Could you check a few things on this model? Use its own coordinates, in mm. A direction names the side the tool comes from. Round coordinates to 2 decimals unless told otherwise and drop trailing zeros. Loops run counter-clockwise (first coordinate to the right, second up) from the corner with the lowest first, then second, coordinate; pieces in that order, holes last. Notation, with made-up numbers: (22.5, 35.5) -> (61.5, 35.5) arc R25 ccw to (61.5, 74.5) -> close; hole circle Ø6 at (4, 80). An arc over 180 degrees is marked (long way). Use CSV: the item, a comma, the result in double quotes. Start each with the question number.
```python
from build123d import *

# Parameters (mm, degrees)
CARRIAGE_PLATE_PROFILE_R   = 5
CARRIAGE_PLATE_PROFILE_R_2 = 3
CARRIAGE_PLATE_5MM_DEPTH   = 5


with BuildPart() as part:
    # Carriage Plate Profile → Carriage Plate 5mm (new body)
    with BuildSketch(Plane.XY):
        with BuildLine():
            Line((-10, -5), (-10, 35))
            ThreePointArc((-10, 35), (-8.535533906, 38.535533906), (-5, 40))
            Line((-5, 40), (5, 40))
            ThreePointArc((5, 40), (8.535533906, 38.535533906), (10, 35))
            Line((10, 35), (10, 30))
            Line((10, 30), (30, 30))
            ThreePointArc((30, 30), (50.922837109, 16.451383494), (75, 10))
            Line((75, 10), (80, 10))
            ThreePointArc((80, 10), (83.535533906, 8.535533906), (85, 5))
            Line((85, 5), (85, -5))
            ThreePointArc((85, -5), (83.535533906, -8.535533906), (80, -10))
            Line((80, -10), (75, -10))
            Line((75, -10), (70, -10))
            ThreePointArc((70, -10), (66.464466094, -8.535533906), (65, -5))
            Line((65, -5), (65, -4))
            ThreePointArc((65, -4), (63.828427125, -1.171572875), (61, 0))
            Line((61, 0), (14, 0))
            ThreePointArc((14, 0), (11.171572875, -1.171572875), (10, -4))
            Line((10, -4), (10, -5))
            ThreePointArc((10, -5), (8.535533906, -8.535533906), (5, -10))
            Line((5, -10), (-5, -10))
            ThreePointArc((-5, -10), (-8.535533906, -8.535533906), (-10, -5))
        make_face()
        Circle(CARRIAGE_PLATE_PROFILE_R, mode=Mode.SUBTRACT)
        with Locations((75, 0)):
            Circle(CARRIAGE_PLATE_PROFILE_R, mode=Mode.SUBTRACT)
        with Locations((0, 30)):
            Circle(CARRIAGE_PLATE_PROFILE_R_2, mode=Mode.SUBTRACT)
    extrude(amount=CARRIAGE_PLATE_5MM_DEPTH)


solid = part.part
```
1. We'd pull the mould along Y, two halves only. Please class faces 4 (the face through (-1.08, -4.88, 2.46)), 5 (the face through (20, 30, 2)), 6 (the face through (11.203, -1.141, 2.465)): pulls with the +Y half, pulls with the -Y half, needs draft (parallel to the pull), parting line crosses it, or undercut.
2. If I drill on L1, parallel to Y at x = 0, z = 1.25; L2, parallel to X at y = 3, z = 3.3; L3, parallel to X at y = 3.5, z = 0.75, over which ranges is the centre line in solid material (lowest first)?
3. Suppose I cut it at D-D (x = 33.5). List the corners of the cut face in (y, z) for me, then the cut area to 3 significant figures.
4. For faces 1 (the face through (10, 33, 2)), 2 (the face through (38, 0, 2)), 3 (the face through (-10, 15, 2)), which set-ups out of +Z, -Z, +X, -X, +Y, -Y let a thin tool reach every point of the face, with its end or its side?
5. Will these pins go through, and if not, where does the flat tip stop? pin 1 (1.5 mm diameter, centred on y = 32.5, z = 2, fed in from +X); pin 2 (3 mm diameter, centred on x = 5, y = 24.5, fed in from -Z); pin 3 (1.5 mm diameter, centred on x = 77.5, z = 3, fed in from +Y); pin 4 (2.5 mm diameter, centred on x = 25, z = 2, fed in from +Y).
6. Suppose I cut it at A-A (x = 0). List the corners of the cut face in (y, z) for me, then the cut area to 3 significant figures.
7. Suppose I cut it at B-B (z = 1.7). List the corners of the cut face in (x, y) for me, then the cut area to 3 significant figures.
8. Suppose I cut it at C-C (y = 12). List the corners of the cut face in (x, z) for me.
Geometry check:
1,face 4,"undercut"
1,face 5,"pulls with the +Y half"
1,face 6,"pulls with the -Y half"
2,L1,"y = -10 to -5, 5 to 27, 33 to 40"
2,L2,"x = -10 to -4, 4 to 71, 79 to 85"
2,L3,"x = -10 to -3.57, 3.57 to 71.43, 78.57 to 85"
3,outline,"(0, 0) -> (27.04, 0) -> (27.04, 5) -> (0, 5) -> close"
3,area,"135 mm²"
4,face 1,"+Z, -Z, +X, +Y"
4,face 2,"+Z, -Z, -Y"
4,face 3,"+Z, -Z, -X, +Y, -Y"
5,pin 1,"stops at x = 10"
5,pin 2,"stops at z = 0"
5,pin 3,"stops at y = 10"
5,pin 4,"stops at y = 30"
6,outline,"(-10, 0) -> (-5, 0) -> (-5, 5) -> (-10, 5) -> close; (5, 0) -> (27, 0) -> (27, 5) -> (5, 5) -> close; (33, 0) -> (40, 0) -> (40, 5) -> (33, 5) -> close"
6,area,"170 mm²"
7,outline,"(-10, -5) arc R5 ccw to (-5, -10) -> (5, -10) arc R5 ccw to (10, -5) -> (10, -4) arc R4 cw to (14, 0) -> (61, 0) arc R4 cw to (65, -4) -> (65, -5) arc R5 ccw to (70, -10) -> (80, -10) arc R5 ccw to (85, -5) -> (85, 5) arc R5 ccw to (80, 10) -> (75, 10) arc R80 cw to (30, 30) -> (10, 30) -> (10, 35) arc R5 ccw to (5, 40) -> (-5, 40) arc R5 ccw to (-10, 35) -> close; hole circle Ø10 at (0, 0); hole circle Ø6 at (0, 30); hole circle Ø10 at (75, 0)"
7,area,"2,460 mm²"
8,outline,"(-10, 0) -> (63.79, 0) -> (63.79, 5) -> (-10, 5) -> close"
